from build123d import *

# Parameters (mm, degrees)
BRACKET_SIDE_PROFILE_SKETCH_R = 9
BRACKET_BODY_41MM_DEPTH       = 20.5
TOP_FACE_CUTS_SKETCH_R        = 6
TOP_FACE_CUTS_SKETCH_W        = 42
TOP_FACE_CUTS_SKETCH_H        = 5
TOP_FACE_CUTS_DEPTH           = 143.425779095
END_SLOT_SKETCH_W             = 12
END_SLOT_SKETCH_H             = 7
END_SLOT_12MM_DEPTH           = 143.425779095
EDGE_CHAMFER_3MM_SIZE         = 3


with BuildPart() as part:
    # Bracket Side Profile Sketch → Bracket Body 41mm (new, symmetric)
    with BuildSketch(Plane.XY):
        with BuildLine():
            Line((0, 0), (-45, 0))
            ThreePointArc((-45, 0), (-47.988718556, 7.130352903), (-55.168386504, 9.998582199))
            Line((-55.168386504, 9.998582199), (-86.000956968, 9.998582199))
            Line((-86.000956968, 9.998582199), (-110, 9.998582199))
            ThreePointArc((-110, 9.998582199), (-131, 30.998582199), (-110, 51.998582199))
            Line((-110, 51.998582199), (-85.996841991, 51.998582199))
            Line((-85.996841991, 51.998582199), (-60, 51.998582199))
            Line((-60, 51.998582199), (-45.996841991, 32))
            Line((-45.996841991, 32), (0, 32))
            Line((0, 32), (0, 0))
        make_face()
        with Locations((-110, 30.998582199)):
            Circle(BRACKET_SIDE_PROFILE_SKETCH_R, mode=Mode.SUBTRACT)
    extrude(amount=BRACKET_BODY_41MM_DEPTH, both=True)

    # Top Face Cuts Sketch → Top Face Cuts (cut, through all)
    with BuildSketch(Plane(origin=(0, 51.998582199, 0), x_dir=(1, 0, 0), z_dir=(0, 1, 0))):
        with Locations(Location((-72.998420995, 0, 0), (0, 0, 270))):
            Circle(TOP_FACE_CUTS_SKETCH_R)
        with Locations(Location((-22.998420995, 0, 0), (0, 0, 270))):
            Circle(TOP_FACE_CUTS_SKETCH_R)
        with Locations((-110, -18)):
            Rectangle(TOP_FACE_CUTS_SKETCH_W, TOP_FACE_CUTS_SKETCH_H)
    extrude(amount=-TOP_FACE_CUTS_DEPTH, mode=Mode.SUBTRACT)

    # End Slot Sketch → End Slot 12mm (cut, through all)
    with BuildSketch(Plane(origin=(0, 0, 0), x_dir=(0, 0, -1), z_dir=(1, 0, 0))):
        with Locations((0, 3.5)):
            Rectangle(END_SLOT_SKETCH_W, END_SLOT_SKETCH_H)
    extrude(amount=-END_SLOT_12MM_DEPTH, mode=Mode.SUBTRACT)

    # Edge Chamfer 3mm
    edge_chamfer_3mm_edges = [part.edges().sort_by_distance(p)[0] for p in [
        (0, 16, -20.5),
        (-74.5, 51.998582199, 20.5),
        (0, 16, 20.5),
    ]]
    chamfer(edge_chamfer_3mm_edges, length=EDGE_CHAMFER_3MM_SIZE)


solid = part.part
Could you check a few things on this model? Use its own coordinates, in mm. A direction names the side the tool comes from. Coordinates: 2 decimals unless noted, no trailing zeros. Loops run counter-clockwise (first coordinate to the right, second up) from the corner with the lowest first, then second, coordinate; pieces in that order, holes last.
1. For faces 4 (the face through (-24, 3, -6)), 5 (the face through (-101, 27, 15.5)), 6 (the face through (-18, 32, 5)), 7 (the face through (-1.5, 16.2, -19)), 8 (the face through (-1.5, 16.2, 19)), which set-ups out of +Z, -Z, +X, -X, +Y, -Y let a thin tool reach every point of the face, with its end or its side?
2. We'd pull the mould along X, two halves only. Please class faces 1 (the face through (-28.856, 19.675, -1.301)), 2 (the face through (-82, 9.999, 0)), 3 (the face through (0, 16, 0)): released by +X, released by -X, zero draft, split by the parting line, or undercut.
3. Imagine slicing it at B-B (y = 35.5). Please give me the cut outline in (x, z), and give its area (3 significant figures).
4. Imagine slicing it at D-D (x = -82). Please give me the cut outline in (y, z).
5. Imagine slicing it at A-A (z = -2.5). Please give me the cut outline in (x, y).
6. For P1, Ø12.5, axis at x = -118.5, y = 41.5, coming from the +Z side; P2, Ø12.5, axis at x = -25.5, z = 4.5, coming from the +Y side; P3, Ø2, axis at y = 43, z = 8, coming from the -X side; P4, Ø11, axis at x = -110, y = 31, coming from the -Z side, each with a flat end and sliding along its axis, tell me the tip position at first contact or that it passes through.
7. Imagine slicing it at C-C (z = 4.5). Please give me the cut outline in (x, y), and give its area (3 significant figures).
8. I need wall thicknesses on L1, parallel to Y at x = -110, z = 5; L2, parallel to X at y = 12.5, z = 0; L3, parallel to Y at x = -6.5, z = -6.5. Which ranges of each line are inside material? Lowest first, please.
Computed values:
1. face 4: +X, -X, -Y
1. face 5: +Z, -X, +Y, -Y
1. face 6: +Z, -Z, +X, +Y
1. face 7: -Z, +X, +Y, -Y
1. face 8: +Z, +X, +Y, -Y
2. face 1: undercut
2. face 2: zero draft
2. face 3: released by +X
3. outline: (-130.51, -20.5) - (-117.79, -20.5) - (-117.79, 15.5) - (-130.51, 15.5) - close; (-102.21, -20.5) - (-48.45, -20.5) - (-48.45, 20.5) - (-89, 20.5) - (-89, 15.5) - (-102.21, 15.5) - close; hole circle Ø12 at (-73, 0)
3. area: 2,480 mm2
4. outline: (10, -20.5) - (52, -20.5) - (52, 17.5) - (49, 20.5) - (10, 20.5) - close
5. outline: (-110, 10) - (-78.45, 10) - (-78.45, 52) - (-110, 52) arc R21 ccw to start; (-67.54, 10) - (-55.17, 10) arc R10 cw to (-47.86, 7) - (-28.45, 7) - (-28.45, 32) - (-46, 32) - (-60, 52) - (-67.54, 52) - close; (-17.54, 7) - (0, 7) - (0, 32) - (-17.54, 32) - close; hole circle Ø18 at (-110, 31)
6. P1: stops at z = 15.5
6. P2: stops at y = 32
6. P3: stops at x = -127.89
6. P4: passes through
7. outline: (-110, 10) - (-76.97, 10) - (-76.97, 52) - (-110, 52) arc R21 ccw to start; (-69.03, 10) - (-55.17, 10) arc R10 cw to (-47.86, 7) - (-26.97, 7) - (-26.97, 32) - (-46, 32) - (-60, 52) - (-69.03, 52) - close; (-19.03, 7) - (0, 7) - (0, 32) - (-19.03, 32) - close; hole circle Ø18 at (-110, 31)
7. area: 3,620 mm2
8. L1: y = 10 to 22, 40 to 52
8. L2: x = -119.94 to -79, -67 to -29, -17 to 0
8. L3: y = 0 to 32
